Geometry check sheet. Reference: the model listing, model coordinates, mm. Face numbers are marked on the shaded views. A direction names the side the tool comes from. Coordinates: 2 decimals unless noted, no trailing zeros. Write each loop counter-clockwise with the first axis right and the second up, starting at its lowest first coordinate (ties: lowest second). Pieces come first, ordered by that corner, then holes. Notation, with made-up numbers: (-39.5, 8) -> (9.5, 8) arc R26 ccw to (9.5, 28) -> close; hole circle Ø4 at (53, 14.25). An arc over 180 degrees is marked (long way). One line per question, with ' | ' between items.
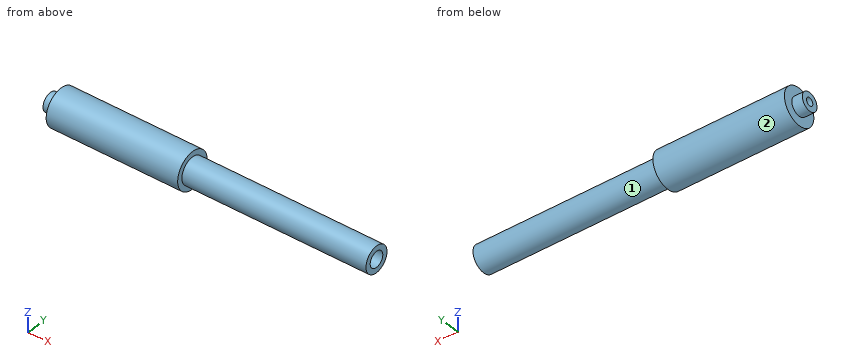
```python
from build123d import *


with BuildPart() as part:
    # Sketch1 → Revolve1 (revolve)
    with BuildSketch(Plane.XY, mode=Mode.PRIVATE) as revolve1_sk:
        Polygon((631.173921275, 208.284534899), (631.173921275, 218.284534899), (281.173921275, 218.284534899), (281.173921275, 228.284534899), (31.173921275, 228.284534899), (31.173921275, 210.784534899), (11.173921275, 210.784534899), (11.173921275, 200.784534899), (41.173921275, 200.784534899), (41.173921275, 218.284534899), (271.173921275, 218.284534899), (271.173921275, 208.284534899), align=None)
    revolve(revolve1_sk.sketch.rotate(Axis((-12.5607058, 193.284534899, 0), (1, 0, 0)), 90), axis=Axis((-12.5607058, 193.284534899, 0), (1, 0, 0)))


solid = part.part
```
(1) Cross-section at B-B (x = 507). Record the cut outline in (y, z).
Answers below:
outline: circle Ø50 at (193.28, 0); hole circle Ø30 at (193.28, 0)
(2) Depth check by flat-ended pin: P1, Ø4, axis at y = 196.5, z = -9.5, coming from the +X side; P2, Ø8, axis at y = 170, z = -23, coming from the +X side; P3, Ø4, axis at x = 502.5, y = 202, coming from the -Z side. Enter the tip coordinate at first touch or a pass-through.
Answers below:
P1: stops at x = 41.17 | P2: stops at x = 281.17 | P3: stops at z = -24.08
(3) Tool access check on the marked faces 1 and 2. Record the directions out of +Z, -Z, +X, -X, +Y, -Y that give a thin tool (end or side, any length) a straight path to the whole face; none if there is none.
Answers below:
face 1: +X | face 2: +X, -X
(4) Material ranges on line 1 (Y direction, x = 33.25, z = 0); line 2 (Y direction, x = 280, z = -1.5); line 3 (Z direction, x = 252, y = 192), recorded low to high.
Answers below:
line 1: y = 158.28 to 185.78, 200.78 to 228.28 | line 2: y = 158.32 to 178.36, 208.21 to 228.25 | line 3: z = -34.98 to -24.97, 24.97 to 34.98
(5) Cross-section at A-A (z = 0). Record the cut outline in (x, y).
Answers below:
outline: (11.17, 175.78) -> (31.17, 175.78) -> (31.17, 158.28) -> (281.17, 158.28) -> (281.17, 168.28) -> (631.17, 168.28) -> (631.17, 178.28) -> (271.17, 178.28) -> (271.17, 168.28) -> (41.17, 168.28) -> (41.17, 185.78) -> (11.17, 185.78) -> close; (11.17, 200.78) -> (41.17, 200.78) -> (41.17, 218.28) -> (271.17, 218.28) -> (271.17, 208.28) -> (631.17, 208.28) -> (631.17, 218.28) -> (281.17, 218.28) -> (281.17, 228.28) -> (31.17, 228.28) -> (31.17, 210.78) -> (11.17, 210.78) -> close
